Job drawing, mm, ordinate dimensions from the low corner. One solid piece. A direction names the side the tool comes from. Round coordinates to 2 decimals unless told otherwise and drop trailing zeros. Write each loop counter-clockwise with the first axis right and the second up, starting at its lowest first coordinate (ties: lowest second). Pieces come first, ordered by that corner, then holes.
1) Saw through at A-A on y = 10. Write the cut outline in (x, z).
2) Drill centre lines: L1, parallel to Z at x = 3.5, y = 4; L2, parallel to Z at x = 7.75, y = 1.75; L3, parallel to Y at x = 6.25, z = 11. Where is each one in solid material? Low to high.
3) Saw through at D-D on z = 18. Write the cut outline in (x, y), and give its area (3 significant figures).
4) Saw through at B-B on x = 6.4. Write the cut outline in (y, z).
5) Which spindle directions (+Z, -Z, +X, -X, +Y, -Y) get a long thin tool onto all of the face, cutting with end or side? Do the marked faces 1 and 2. Say none if no direction does.
6) Flat gauge pins, fed straight in: pin 1 (5 mm diameter, centred on y = 7.5, z = 5.5, fed in from -X); pin 2 (3 mm diameter, centred on x = 5, y = 6.5, fed in from -Z); pin 3 (3 mm diameter, centred on x = 10.5, y = 11, fed in from -Z); pin 4 (2 mm diameter, centred on x = 4, z = 15.5, fed in from -Y) (3 decimals). Where does each tip first touch, or does it go through?
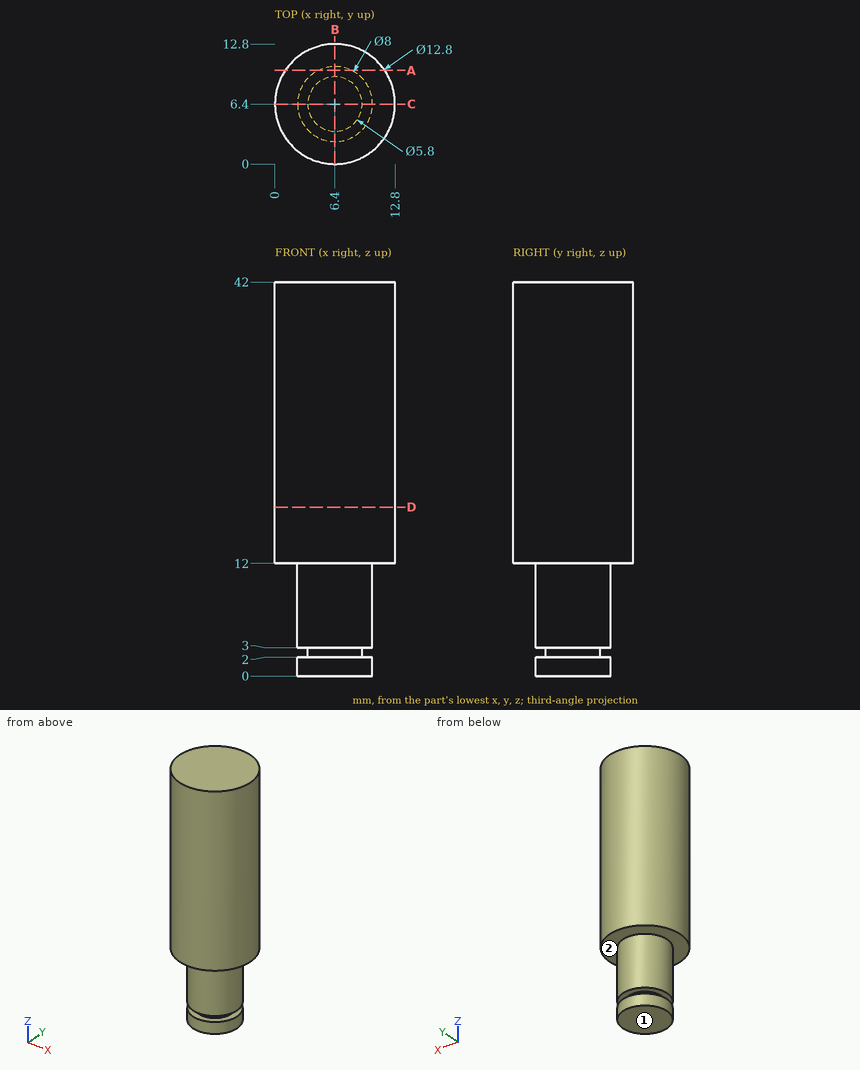
Completed:
1. outline: (1.11, 12) - (4.66, 12) - (4.66, 3) - (8.14, 3) - (8.14, 12) - (11.69, 12) - (11.69, 42) - (1.11, 42) - close; (4.66, 0) - (8.14, 0) - (8.14, 2) - (4.66, 2) - close
2. L1: z = 0 to 2, 3 to 42
2. L2: z = 12 to 42
2. L3: y = 2.4 to 10.4
3. outline: circle Ø12.8 at (6.4, 6.4)
3. area: 129 mm2
4. outline: (0, 12) - (2.4, 12) - (2.4, 3) - (3.5, 3) - (3.5, 2) - (2.4, 2) - (2.4, 0) - (10.4, 0) - (10.4, 2) - (9.3, 2) - (9.3, 3) - (10.4, 3) - (10.4, 12) - (12.8, 12) - (12.8, 42) - (0, 42) - close
5. face 1: -Z, +X, -X, +Y, -Y
5. face 2: -Z
6. pin 1: stops at x = 2.4
6. pin 2: stops at z = 0
6. pin 3: stops at z = 12
6. pin 4: stops at y = 0.155
